Read the model definition and answer for the solid it produces. Units are mm, in the model's axes. Face numbers are marked on the shaded views. A direction names the side the tool comes from. Give positions to 0.01 mm unless a question says otherwise; leave off trailing zeros. Order: outer loops, then holes, each group sorted by start corner. A loop starts at its lowest first (then second) coordinate and runs counter-clockwise, first axis right, second up.
Item 1: Given pin 1 Ø1 at (x, z) = (6, 21.5) entering from +Y; pin 2 Ø24 at (x, y) = (0, 0) entering from +Z; pin 3 Ø6 at (x, y) = (-23.57, -23.57) entering from +Z, each flat-ended and moving along its own axis, determine where each tip first touches the part or whether it passes through.
Item 2: A cutting plane is placed at C-C (y = 2). Write down the section's boundary in (x, z).
Item 3: A cutting plane is placed at A-A (x = 0). Write down the section's boundary in (y, z).
Item 4: A cutting plane is placed at D-D (x = -12). Write down the section's boundary in (y, z).
Item 5: Find the intervals of material crossed by line 1 along Y through (x, z) = (23.57, 1.75); line 2 along X through (y, z) = (23.57, 1.15); line 3 along X through (y, z) = (23, 1), in increasing order.
Item 6: A cutting plane is placed at B-B (y = 23.57). Write down the section's boundary in (x, z).
Item 7: Which of the six approach directions +Z, -Z, +X, -X, +Y, -Y give full straight-line access (tool end or side, diameter ignored) to the marked faces 1, 2 and 3?
from build123d import *

# Parameters (mm, degrees)
SKETCH_1_W               = 70
SKETCH_1_H               = 65
EXTRUDE_1_DEPTH          = 5
CUT_EXTRUDE_2_DEPTH      = 49.023431781
CUT_EXTRUDE_2_DEPTH_BACK = 49.023431781
SKETCH_3_R               = 2.55
SKETCH_4_W               = 70
SKETCH_4_H               = 5
EXTRUDE_2_DEPTH          = 90
FILLET_1_R               = 1
FILLET_2_R               = 1
CUT_EXTRUDE_START        = -5
SKETCH_5_R               = 20
CUT_EXTRUDE_3_DEPTH      = 2
CUT_EXTRUDE_4_DEPTH      = 104.659297702
CUT_EXTRUDE_4_DEPTH_BACK = 104.659297702
SKETCH_6_R               = 5


with BuildPart() as part:
    # 草图1 → 凸台-拉伸1 (new body)
    with BuildSketch(Plane.XY):
        Rectangle(SKETCH_1_W, SKETCH_1_H)
    extrude(amount=EXTRUDE_1_DEPTH)

    # 草图3 → 切除-拉伸2 (cut, two sides: drawn at the far end of the back side and taken through both)
    with BuildSketch(Plane.XY.offset(5).offset(-CUT_EXTRUDE_2_DEPTH_BACK)):
        with Locations((-23.57, 23.57)):
            Circle(SKETCH_3_R)
        with Locations((23.57, 23.57)):
            Circle(SKETCH_3_R)
        with Locations((23.57, -23.57)):
            Circle(SKETCH_3_R)
        with Locations((-23.57, -23.57)):
            Circle(SKETCH_3_R)
    extrude(amount=CUT_EXTRUDE_2_DEPTH + CUT_EXTRUDE_2_DEPTH_BACK, mode=Mode.SUBTRACT)

    # 草图4 → 凸台-拉伸2 (add)
    with BuildSketch(Plane.XY.offset(5)):
        with Locations((0, -30)):
            Rectangle(SKETCH_4_W, SKETCH_4_H)
    extrude(amount=EXTRUDE_2_DEPTH)

    # 圆角1
    fillet_1_edges = [part.edges().sort_by_distance(p)[0] for p in [
        (0, -27.5, 5),
    ]]
    fillet(fillet_1_edges, radius=FILLET_1_R)

    # 圆角2
    fillet_2_edges = [part.edges().sort_by_distance(p)[0] for p in [
        (0, -32.5, 0),
    ]]
    fillet(fillet_2_edges, radius=FILLET_2_R)

    # 草图5 → 切除-拉伸3 (cut)
    with BuildSketch(Plane(origin=(0, 0, 0), x_dir=(-1, 0, 0), z_dir=(0, 0, -1)).offset(CUT_EXTRUDE_START)):
        with Locations(Location((0, 0, 0), (0, 0, 180))):
            Circle(SKETCH_5_R)
    extrude(amount=CUT_EXTRUDE_3_DEPTH, mode=Mode.SUBTRACT)

    # 草图6 → 切除-拉伸4 (cut, two sides: drawn at the far end of the back side and taken through both)
    with BuildSketch(Plane.XY.offset(3).offset(-CUT_EXTRUDE_4_DEPTH_BACK)):
        Circle(SKETCH_6_R)
    extrude(amount=CUT_EXTRUDE_4_DEPTH + CUT_EXTRUDE_4_DEPTH_BACK, mode=Mode.SUBTRACT)


solid = part.part
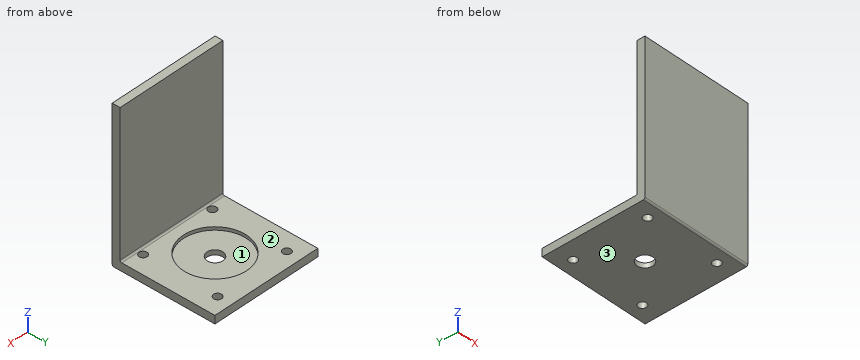
Response values:
1. pin 1: stops at y = -27.5
1. pin 2: stops at z = 3
1. pin 3: stops at z = 5
2. outline: (-35, 0) - (-4.58, 0) - (-4.58, 3) - (-19.9, 3) - (-19.9, 5) - (-35, 5) - close; (4.58, 0) - (35, 0) - (35, 5) - (19.9, 5) - (19.9, 3) - (4.58, 3) - close
3. outline: (-32.5, 1) arc R1 ccw to (-31.5, 0) - (-5, 0) - (-5, 3) - (-20, 3) - (-20, 5) - (-26.5, 5) arc R1 cw to (-27.5, 6) - (-27.5, 95) - (-32.5, 95) - close; (5, 0) - (32.5, 0) - (32.5, 5) - (20, 5) - (20, 3) - (5, 3) - close
4. outline: (-32.5, 1) arc R1 ccw to (-31.5, 0) - (32.5, 0) - (32.5, 5) - (16, 5) - (16, 3) - (-16, 3) - (-16, 5) - (-26.5, 5) arc R1 cw to (-27.5, 6) - (-27.5, 95) - (-32.5, 95) - close
5. line 1: y = -32.5 to -26.12, -21.02 to 21.02, 26.12 to 32.5
5. line 2: x = -35 to -26.12, -21.02 to 21.02, 26.12 to 35
5. line 3: x = -35 to -26.06, -21.08 to 21.08, 26.06 to 35
6. outline: (-35, 0) - (-26.12, 0) - (-26.12, 5) - (-35, 5) - close; (-21.02, 0) - (21.02, 0) - (21.02, 5) - (-21.02, 5) - close; (26.12, 0) - (35, 0) - (35, 5) - (26.12, 5) - close
7. face 1: +Z
7. face 2: +Z, +X, -X, +Y
7. face 3: -Z, +X, -X, +Y, -Y
